Source: CAD feature listing. Evaluate the final solid. Frame: model axes, mm. A direction names the side the tool comes from. Give positions to 0.01 mm unless a question says otherwise; leave off trailing zeros. Order: outer loops, then holes, each group sorted by start corner. A loop starts at its lowest first (then second) coordinate and runs counter-clockwise, first axis right, second up.
from build123d import *

# Parameters (mm, degrees)
BOSS_EXTRUDE1_DEPTH = 10
SKETCH4_R           = 26.75
SKETCH4_R_2         = 12
CUT_EXTRUDE1_DEPTH  = 1.25
CUT_EXTRUDE1_DRAFT  = -60
CHAMFER2_SIZE       = 0.888888889


with BuildPart() as part:
    # Sketch3 → Boss-Extrude1 (new body)
    with BuildSketch(Plane(origin=(0, 0, 0), x_dir=(0, 0, -1), z_dir=(1, 0, 0))):
        Polygon((12, 6.92820323), (0, 13.856406461), (-12, 6.92820323), (-12, -6.92820323), (0, -13.856406461), (12, -6.92820323), align=None)
    extrude(amount=BOSS_EXTRUDE1_DEPTH)


with BuildPart() as cut_extrude1_tool:
    # Sketch4 → Cut-Extrude1 (with draft: the straight prism first)
    with BuildSketch(Plane.ZY):
        Circle(SKETCH4_R)
        Circle(SKETCH4_R_2, mode=Mode.SUBTRACT)
    extrude(amount=-CUT_EXTRUDE1_DEPTH)
    # Cut-Extrude1: the draft: its side faces are tilted about the plane it starts from
    cut_extrude1_sides = [cut_extrude1_tool.faces().sort_by_distance(p)[0] for p in [
        (0.625, 0, -26.75),
        (0.625, 0, -12),
    ]]
    draft(cut_extrude1_sides, Plane.ZY, CUT_EXTRUDE1_DRAFT)


with BuildPart() as part_1:
    add(part.part)

    # Cut-Extrude1: cut by cut_extrude1_tool
    add(cut_extrude1_tool.part, mode=Mode.SUBTRACT)

    # Sketch5 → Revolve1 (revolve)
    with BuildSketch(Plane.XY, mode=Mode.PRIVATE) as revolve1_sk:
        with BuildLine():
            Line((10.85, 8), (150, 8))
            Line((150, 8), (150, 0))
            Line((150, 0), (10, 0))
            Line((10, 0), (10, 8.85))
            ThreePointArc((10, 8.85), (10.248959236, 8.248959236), (10.85, 8))
        make_face()
    revolve(revolve1_sk.sketch.rotate(Axis((10, 0, 0), (1, 0, 0)), 90), axis=Axis((10, 0, 0), (1, 0, 0)))

    # Chamfer2
    chamfer2_edges = [part_1.edges().sort_by_distance(p)[0] for p in [
        (150, 0, -8),
    ]]
    chamfer(chamfer2_edges, length=CHAMFER2_SIZE)

    # Sketch7 → Cut-Revolve1 (revolve, cut)
    with BuildSketch(Plane.XY, mode=Mode.PRIVATE) as cut_revolve1_sk:
        Polygon((10, 11.145), (9.2, 11.945), (9.2, 26.75), (10, 26.75), align=None)
    revolve(cut_revolve1_sk.sketch.rotate(Axis((0, 0, 0), (1, 0, 0)), 90), axis=Axis((0, 0, 0), (1, 0, 0)), mode=Mode.SUBTRACT)


solid = part_1.part
1) Section query A-A on x = 29. Output: boundary loops of the cut face in (y, z), and give its area (3 significant figures).
Checks:
outline: circle Ø16 at (0, 0)
area: 201 mm2
2) First-contact query: pin 1 Ø4 at (y, z) = (1.5, -9) entering from -X; pin 2 Ø8 at (x, z) = (62.5, -6.5) entering from -Y; pin 3 Ø5 at (x, y) = (74.5, 8) entering from +Z; pin 4 Ø6 at (x, y) = (63.5, -3.5) entering from +Z. Flat tips, straight axial feed; report the tip coordinate or a pass-through.
Checks:
pin 1: stops at x = 0
pin 2: stops at y = -7.6
pin 3: stops at z = 5.81
pin 4: stops at z = 7.98
3) Ray query, L1, parallel to X at y = 6.25, z = 7.75; L2, parallel to Y at x = 100, z = 0.5; L3, parallel to Y at x = 64, z = -3. Return the intervals inside material, ascending.
Checks:
L1: x = 0 to 10
L2: y = -7.98 to 7.98
L3: y = -7.42 to 7.42
4) Reachability of faces 1 (the face through (10, 9, -1)), 2 (the face through (0.256, 6.195, 10.791)) from +Z, -Z, +X, -X, +Y, -Y: full face, straight path, thin tool, end or side. Return the list, or none.
Checks:
face 1: +X
face 2: +Z, -X, +Y
